Geometry check sheet. Reference: the model listing, model coordinates, mm. Face numbers are marked on the shaded views. A direction names the side the tool comes from. Coordinates: 2 decimals unless noted, no trailing zeros. Write each loop counter-clockwise with the first axis right and the second up, starting at its lowest first coordinate (ties: lowest second). Pieces come first, ordered by that corner, then holes. Notation, with made-up numbers: (70.25, -3) - (118.25, -3) arc R10 cw to (118.25, 8) - close; hole circle Ø2 at (-24, 3). An arc over 180 degrees is marked (long way). Answer as a JSON object with one key per item and string values. Group by question number.
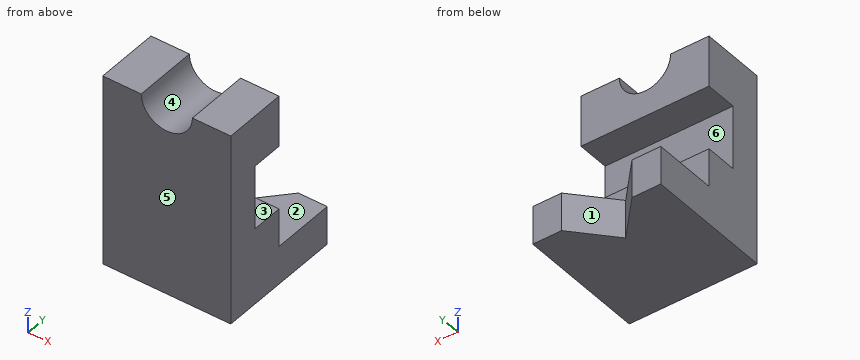
from build123d import *

# Parameters (mm, degrees)
BASE_BODY_DEPTH        = 60
UPRIGHT_PROFILE_W      = 40
UPRIGHT_PROFILE_H      = 20
UPRIGHT_BLOCK_DEPTH    = 12
STEP_CUT_PROFILE_W     = 20
STEP_CUT_PROFILE_H     = 20
STEP_CUT_DEPTH         = 60
HALF_ROUND_NOTCH_DEPTH = 60
CROSS_SLOT_PROFILE_W   = 20
CROSS_SLOT_PROFILE_H   = 10
CROSS_SLOT_DEPTH       = 60
ANGLED_NOTCH_DEPTH     = 60


with BuildPart() as part:
    # Base Profile → Base Body (new body)
    with BuildSketch(Plane.XY):
        Polygon((0, 0), (60, 0), (60, 20), (16, 20), (0, 20), align=None)
    extrude(amount=BASE_BODY_DEPTH)

    # Upright Profile → Upright Block (add)
    with BuildSketch(Plane(origin=(0, 0, 0), x_dir=(-1, 0, 0), z_dir=(0, 0, -1))):
        with Locations((-40, 30)):
            Rectangle(UPRIGHT_PROFILE_W, UPRIGHT_PROFILE_H)
    extrude(amount=-UPRIGHT_BLOCK_DEPTH)

    # Step Cut Profile → Step Cut (cut)
    with BuildSketch(Plane(origin=(0, 0, 0), x_dir=(-1, 0, 0), z_dir=(0, 0, -1))):
        with Locations((-10, 10)):
            Rectangle(STEP_CUT_PROFILE_W, STEP_CUT_PROFILE_H)
    extrude(amount=-STEP_CUT_DEPTH, mode=Mode.SUBTRACT)

    # Half-Round Notch Profile → Half-Round Notch (cut)
    with BuildSketch(Plane(origin=(0, 20, 0), x_dir=(1, 0, 0), z_dir=(0, 1, 0))):
        with BuildLine():
            Line((32, -60), (48, -60))
            ThreePointArc((48, -60), (40, -52), (32, -60))
        make_face()
    extrude(amount=-HALF_ROUND_NOTCH_DEPTH, mode=Mode.SUBTRACT)

    # Cross Slot Profile → Cross Slot (cut)
    with BuildSketch(Plane(origin=(60, 0, 0), x_dir=(0, 0, -1), z_dir=(1, 0, 0))):
        with Locations((-34, 15)):
            Rectangle(CROSS_SLOT_PROFILE_W, CROSS_SLOT_PROFILE_H)
    extrude(amount=-CROSS_SLOT_DEPTH, mode=Mode.SUBTRACT)

    # Angled Notch Profile → Angled Notch (cut)
    with BuildSketch(Plane.XY.offset(12)):
        Polygon((40, 40), (51, 40), (40, 28), (29, 40), align=None)
    extrude(amount=-ANGLED_NOTCH_DEPTH, mode=Mode.SUBTRACT)


solid = part.part
(1) Section check A-A (y = 37). Record the cut outline in (x, z), and give its area (3 significant figures).
(2) Material ranges on L1, parallel to Z at x = 48, y = 20.5; L2, parallel to Y at x = 42.5, z = 50.5; L3, parallel to Y at x = 53, z = 33, recorded low to high. Write a range as [from, to].
(3) Gauge pin test, flat ends, axial feed: pin 1 (8 mm diameter, centred on x = 53, z = 16.5, fed in from +Y); pin 2 (3 mm diameter, centred on x = 42.5, y = 12.5, fed in from +Z); pin 3 (16 mm diameter, centred on x = 31.5, y = 33, fed in from +Z). Record the tip position at first contact, or that the pin passes through.
(4) Set-up check for the marked faces 1, 2 and 3: record each of +Z, -Z, +X, -X, +Y, -Y from which the full face is reachable in a straight line by a thin tool's end or side.
(5) Section check B-B (x = 27). Record the cut outline in (y, z), and give its area (3 significant figures).
(6) Section check C-C (y = 5). Record the cut outline in (x, z), and give its area (3 significant figures).
(7) Draft check along Z on the marked faces 4, 5 and 6. Enter one of: +Z half, -Z half, draft (parallel to the pull), parting line (faces both ways), or undercut.
(8) Section check D-D (z = 36.5). Record the cut outline in (x, y), and give its area (3 significant figures).
Conclusion:
{
 "1": {"outline": "(20, 0) - (31.75, 0) - (31.75, 12) - (20, 12) - close; (48.25, 0) - (60, 0) - (60, 12) - (48.25, 12) - close", "area": "282 mm^2"},
 "2": {"L1": "z = [0, 12]", "L2": "y = [0, 20]", "L3": "y = [0, 10]"},
 "3": {"pin 1": "stops at y = 20", "pin 2": "stops at z = 53.07", "pin 3": "stops at z = 12"},
 "4": {"face 1": "+Z, -Z, +Y", "face 2": "+Z, +X, -X, +Y", "face 3": "+X, -X, +Y"},
 "5": {"outline": "(0, 0) - (40, 0) - (40, 12) - (20, 12) - (20, 24) - (10, 24) - (10, 44) - (20, 44) - (20, 60) - (0, 60) - close", "area": "1,240 mm^2"},
 "6": {"outline": "(20, 0) - (60, 0) - (60, 60) - (48, 60) arc R8 cw to (32, 60) - (20, 60) - close", "area": "2,300 mm^2"},
 "7": {"face 4": "+Z half", "face 5": "draft", "face 6": "undercut"},
 "8": {"outline": "(20, 0) - (60, 0) - (60, 10) - (20, 10) - close", "area": "400 mm^2"}
}
